Design review of the part built by this model. Coordinates are the model's own, in mm. Face numbers are marked on the shaded views. A direction names the side the tool comes from. Give positions to 0.01 mm unless a question says otherwise; leave off trailing zeros. Write each loop counter-clockwise with the first axis right and the second up, starting at its lowest first coordinate (ties: lowest second). Pieces come first, ordered by that corner, then holes. Notation, with made-up numbers: M 12.25,30 L 60.25,30 A7 cw 60.25,36 Z; hole C 34,77.5 d9. An arc over 180 degrees is marked long. Answer in a Markdown table with one row per item.
```python
from build123d import *

# Parameters (mm, degrees)
BASE_PLATE_SKETCH_R     = 6
BASE_PLATE_DEPTH        = 15
INCLINED_ARM_SKETCH_R   = 15
INCLINED_ARM_SKETCH_R_2 = 6.5
INCLINED_ARM_DEPTH      = 15
LUG_WITH_BORE_REACH     = 118.221
LUG_SKETCH_R            = 15


with BuildPart() as part:
    # Base Plate Sketch → Base Plate (new body)
    with BuildSketch(Plane(origin=(0, 0, 0), x_dir=(1, 0, 0), z_dir=(0, 1, 0))):
        with BuildLine():
            Line((-50, 55), (50, 55))
            ThreePointArc((50, 55), (60.606601718, 50.606601718), (65, 40))
            Line((65, 40), (65, -40))
            ThreePointArc((65, -40), (60.606601718, -50.606601718), (50, -55))
            Line((50, -55), (-50, -55))
            ThreePointArc((-50, -55), (-60.606601718, -50.606601718), (-65, -40))
            Line((-65, -40), (-65, 40))
            ThreePointArc((-65, 40), (-60.606601718, 50.606601718), (-50, 55))
        make_face()
        with Locations(Location((-50, 35, 0), (0, 0, 270))):
            Circle(BASE_PLATE_SKETCH_R, mode=Mode.SUBTRACT)
        with Locations(Location((-50, -35, 0), (0, 0, 270))):
            Circle(BASE_PLATE_SKETCH_R, mode=Mode.SUBTRACT)
        with Locations(Location((50, -35, 0), (0, 0, 90))):
            Circle(BASE_PLATE_SKETCH_R, mode=Mode.SUBTRACT)
        with Locations(Location((50, 35, 0), (0, 0, 90))):
            Circle(BASE_PLATE_SKETCH_R, mode=Mode.SUBTRACT)
    extrude(amount=BASE_PLATE_DEPTH)

    # Lug Sketch → Lug with Bore (add, up to next)
    with BuildSketch(Plane(origin=(15.245190528, 26.405444566, 0), x_dir=(0.8660254037844417, -0.4999999999999947, 0), z_dir=(-0.4999999999999947, -0.8660254037844417, 0)), mode=Mode.PRIVATE) as lug_with_bore_sk1:
        with BuildLine():
            ThreePointArc((-12.905713736, 7.5), (-61.754193771, 0), (-12.905713736, -7.5))
            Line((-12.905713736, -7.5), (48.791651246, -7.5))
            Line((48.791651246, -7.5), (48.791651246, 7.5))
            Line((48.791651246, 7.5), (-12.905713736, 7.5))
        make_face()
        with Locations(Location((-36.754193771, 0, 0), (0, 0, 180))):
            Circle(LUG_SKETCH_R, mode=Mode.SUBTRACT)
    lug_with_bore_tool1 = extrude(lug_with_bore_sk1.sketch, amount=LUG_WITH_BORE_REACH, mode=Mode.PRIVATE) - part.part


with BuildPart() as body_2:
    # Inclined Arm Sketch → Inclined Arm (new body)
    with BuildSketch(Plane(origin=(22.745190528, 39.395825623, 0), x_dir=(-0.8660254037844417, 0.4999999999999947, 0), z_dir=(0.4999999999999947, 0.8660254037844417, 0))):
        with BuildLine():
            Line((-4.476862485, 17.5), (-48.791651246, 17.5))
            Line((-48.791651246, 17.5), (-48.791651246, -17.5))
            Line((-48.791651246, -17.5), (-4.476862485, -17.5))
            ThreePointArc((-4.476862485, -17.5), (2.069674222, -19.003968837), (7.303439302, -23.214285714))
            ThreePointArc((7.303439302, -23.214285714), (11.430063197, -27.657519966), (16.21887561, -31.37755102))
            ThreePointArc((16.21887561, -31.37755102), (22.091371242, -38.774247477), (22.379471059, -48.214285714))
            ThreePointArc((22.379471059, -48.214285714), (36.754193771, -67.5), (51.128916484, -48.214285714))
            ThreePointArc((51.128916484, -48.214285714), (51.4170163, -38.774247477), (57.289511932, -31.37755102))
            ThreePointArc((57.289511932, -31.37755102), (64.411713737, 25.324130574), (7.303439302, 23.214285714))
            ThreePointArc((7.303439302, 23.214285714), (2.069674222, 19.003968837), (-4.476862485, 17.5))
        make_face()
        with Locations((36.754193771, 0)):
            Circle(INCLINED_ARM_SKETCH_R, mode=Mode.SUBTRACT)
        with Locations((36.754193771, -52.5)):
            Circle(INCLINED_ARM_SKETCH_R_2, mode=Mode.SUBTRACT)
    extrude(amount=-INCLINED_ARM_DEPTH)


with BuildPart() as part_1:
    add(part.part)

    add(body_2.part)  # Lug with Bore merges body 2
    add(lug_with_bore_tool1.solids().sort_by_distance((3.499955, 33.18656, 0))[0])


solid = part_1.part
```
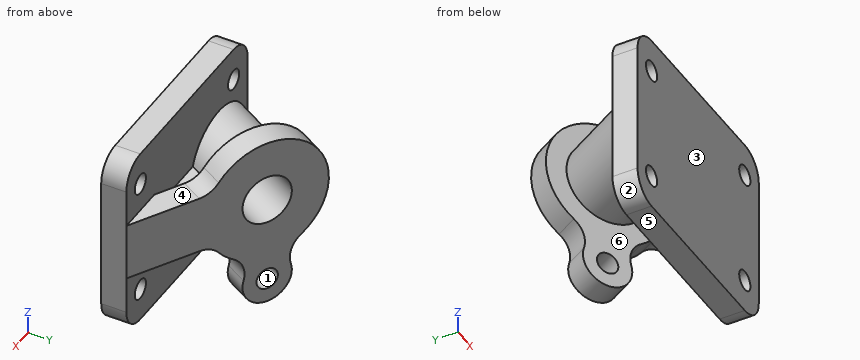
1) The part is to be moulded in two halves that separate along X. For the marked faces 1, 2 and 3, say which applies: released by +X, released by -X, zero draft, split by the parting line, or undercut.
Geometry says:
| item | result |
|---|---|
| face 1 | undercut |
| face 2 | released by -X |
| face 3 | zero draft |
2) Insertion check: P1, Ø1, axis at y = 59.5, z = 18.5, coming from the +X side; P2, Ø9, axis at x = 21.5, y = 20, coming from the -Z side; P3, Ø11, axis at x = 46, y = 27.5, coming from the +Z side; P4, Ø15.5, axis at x = 50, z = -35, coming from the -Y side. Each pin has a flat end and moves straight along its axis. Give the tip position at first contact, or say it passes through.
Geometry says:
| item | result |
|---|---|
| P1 | x = -11.21 |
| P2 | z = -17.5 |
| P3 | z = 17.5 |
| P4 | y = 0 |
3) Add section C-C (z = -35). Write out the cut boundary in (x, y).
Geometry says:
| item | result |
|---|---|
| outline | M -65,0 L -56,0 L -56,15 L -65,15 Z; M -44,0 L 44,0 L 44,15 L -44,15 Z; M -31.04,53.13 L -2.13,36.43 L 5.37,49.42 L -23.54,66.12 Z; M 56,0 L 65,0 L 65,15 L 56,15 Z |
4) For the marked faces 4, 5 and 6, list the 3-axis set-ups (+Z, -Z, +X, -X, +Y, -Y) from which the entire face can be reached by the end or side of a thin tool; tool diameter is ignored.
Geometry says:
| item | result |
|---|---|
| face 4 | +Z, +X |
| face 5 | -Z, +X, -X, -Y |
| face 6 | none |
5) To check wall thickness, follow probe 1 along Z at (x, y) = (50, 4); probe 2 along X at (y, z) = (9, -35); probe 3 along Z at (x, y) = (48.5, 6.5). State the ranges of each line that lie inside material, in increasing order. Write a range as [from, to].
Geometry says:
| item | result |
|---|---|
| probe 1 | [-55, -41], [-29, 29], [41, 55] |
| probe 2 | [-65, -56], [-44, 44], [56, 65] |
| probe 3 | [-55, -40.81], [-29.19, 29.19], [40.81, 55] |
6) Add section A-A (z = 35). Write out the cut boundary in (x, y), and give its area (3 significant figures).
Geometry says:
| item | result |
|---|---|
| outline | M -65,0 L -56,0 L -56,15 L -65,15 Z; M -44,0 L 44,0 L 44,15 L -44,15 Z; M -28.24,51.51 L -4.93,38.05 L 2.57,51.04 L -20.74,64.5 Z; M 56,0 L 65,0 L 65,15 L 56,15 Z |
| area | 1,990 mm^2 |
7) Add section D-D (z = 9.5). Write out the cut boundary in (x, y), and give its area (3 significant figures).
Geometry says:
| item | result |
|---|---|
| outline | M -65,0 L 65,0 L 65,15 L 0.97,51.97 L -20.38,15 L -47.18,15 L -19.14,63.58 L -40.5,75.91 L -48,62.92 L -36.61,56.34 L -60.48,15 L -65,15 Z; hole M -7.08,15 L 35,15 L 3.44,33.22 Z |
| area | 4,030 mm^2 |
8) Add section B-B (y = 6). Write out the cut boundary in (x, z).
Geometry says:
| item | result |
|---|---|
| outline | M -65,-40 A15 ccw -50,-55 L 50,-55 A15 ccw 65,-40 L 65,40 A15 ccw 50,55 L -50,55 A15 ccw -65,40 Z; hole C -50,-35 d12; hole C -50,35 d12; hole C 50,-35 d12; hole C 50,35 d12 |
